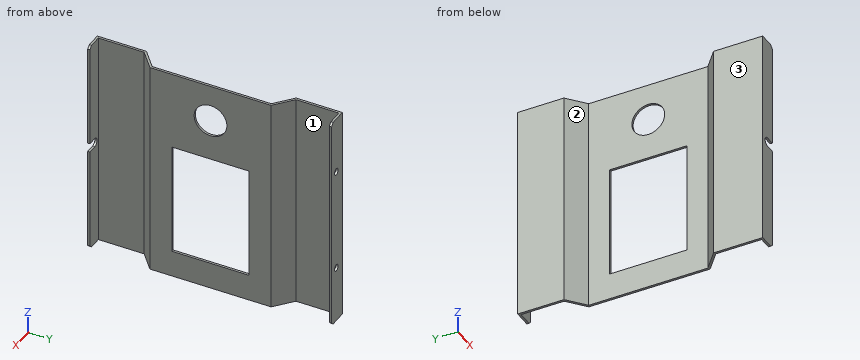
```python
from build123d import *

# Parameters (mm, degrees)
EXTRUDE_THIN1_DEPTH = 73.5
SKETCH2_W           = 76
SKETCH2_H           = 52
CUT_EXTRUDE1_DEPTH  = 10
CHAMFER1_SIZE       = 2
CUT_EXTRUDE3_DEPTH  = 5
SKETCH7_R           = 11
CUT_EXTRUDE4_DEPTH  = 10
SKETCH8_R           = 2.25
CUT_EXTRUDE5_DEPTH  = 10


with BuildPart() as part:
    # Sketch1 → Extrude-Thin1 (new, symmetric)
    with BuildSketch(Plane.XY):
        Polygon((12, 0), (0, 0), (0, 33), (12, 43.248968226), (12, 123.248968226), (0, 133.497936451), (0, 164.497936451), (13.5, 164.497936451), (13.5, 162.997936451), (1.5, 162.997936451), (1.5, 134.189445923), (13.5, 123.940477697), (13.5, 42.557458754), (1.5, 32.308490528), (1.5, 1.5), (12, 1.5), align=None)
    extrude(amount=EXTRUDE_THIN1_DEPTH, both=True)

    # Sketch2 → Cut-Extrude1 (cut)
    with BuildSketch(Plane.ZY.offset(-12)):
        with Locations((-17.5, 83.248968226)):
            Rectangle(SKETCH2_W, SKETCH2_H)
    extrude(amount=-CUT_EXTRUDE1_DEPTH, mode=Mode.SUBTRACT)

    # Chamfer1
    chamfer1_edges = [part.edges().sort_by_distance(p)[0] for p in [
        (13.5, 163.747936451, -73.5),
        (12, 0.75, -73.5),
        (13.5, 163.747936451, 73.5),
        (12, 0.75, 73.5),
    ]]
    chamfer(chamfer1_edges, length=CHAMFER1_SIZE)

    # Sketch6 → Cut-Extrude3 (cut)
    with BuildSketch(Plane.XZ):
        with BuildLine():
            Line((6, 3), (12, 3))
            ThreePointArc((12, 3), (15, 0), (12, -3))
            Line((12, -3), (6, -3))
            ThreePointArc((6, -3), (3, 0), (6, 3))
        make_face()
    extrude(amount=-CUT_EXTRUDE3_DEPTH, mode=Mode.SUBTRACT)

    # Sketch7 → Cut-Extrude4 (cut)
    with BuildSketch(Plane.ZY.offset(-12)):
        with Locations(Location((48.5, 83.248968226, 0), (0, 0, 270))):
            Circle(SKETCH7_R)
    extrude(amount=-CUT_EXTRUDE4_DEPTH, mode=Mode.SUBTRACT)

    # Sketch8 → Cut-Extrude5 (cut)
    with BuildSketch(Plane(origin=(0, 164.497936451, 0), x_dir=(1, 0, 0), z_dir=(0, 1, 0))):
        with Locations(Location((7.5, 35, 0), (0, 0, 180))):
            Circle(SKETCH8_R)
    cut_extrude5 = extrude(amount=-CUT_EXTRUDE5_DEPTH, mode=Mode.SUBTRACT)

    # Mirror1: Cut-Extrude5 across plane
    add(cut_extrude5.mirror(Plane.XY), mode=Mode.SUBTRACT)


solid = part.part
```
Build history of the part. All positions in model axes, mm. Face numbers are marked on the shaded views. A direction names the side the tool comes from. Give positions to 0.01 mm unless a question says otherwise; leave off trailing zeros. Loops run counter-clockwise (first coordinate to the right, second up) from the corner with the lowest first, then second, coordinate; pieces in that order, holes last.
1) 3-axis set-ups, long thin cutter, end or side, ignore diameter. For the marked faces 1, 2 and 3: which of +Z, -Z, +X, -X, +Y, -Y reach the whole face in a straight line?
Values follow:
face 1: +Z, -Z, +X
face 2: +Z, -Z, -X
face 3: +Z, -Z, -X, +Y, -Y
2) Band-saw the part on B-B on y = 61.5. List the corners of the cut face in (x, z), then the cut area to 4 significant figures.
Values follow:
outline: (12, -73.5) - (13.5, -73.5) - (13.5, -55.5) - (12, -55.5) - close; (12, 20.5) - (13.5, 20.5) - (13.5, 73.5) - (12, 73.5) - close
area: 106.5 mm2
3) Probe line 1 along Z through (x, y) = (7.5, 163.85); line 2 along Y through (x, z) = (4.5, 1); line 3 along Y through (x, z) = (2, -38). List the from-to ranges inside material, lowest first.
Values follow:
line 1: z = -73.5 to -37.25, -32.75 to 32.75, 37.25 to 73.5
line 2: y = 34.87 to 36.84, 129.65 to 131.63, 163 to 164.5
line 3: y = 0 to 1.5, 32.74 to 34.71, 131.79 to 133.76, 163 to 164.5
4) Band-saw the part on A-A on z = 0. List the corners of the cut face in (x, y).
Values follow:
outline: (0, 0) - (3, 0) - (3, 1.5) - (1.5, 1.5) - (1.5, 32.31) - (13.5, 42.56) - (13.5, 57.25) - (12, 57.25) - (12, 43.25) - (0, 33) - close; (0, 133.5) - (12, 123.25) - (12, 109.25) - (13.5, 109.25) - (13.5, 123.94) - (1.5, 134.19) - (1.5, 163) - (13.5, 163) - (13.5, 164.5) - (0, 164.5) - close
5) Band-saw the part on D-D on z = 24.5. List the corners of the cut face in (x, y).
Values follow:
outline: (0, 0) - (12, 0) - (12, 1.5) - (1.5, 1.5) - (1.5, 32.31) - (13.5, 42.56) - (13.5, 123.94) - (1.5, 134.19) - (1.5, 163) - (13.5, 163) - (13.5, 164.5) - (0, 164.5) - (0, 133.5) - (12, 123.25) - (12, 43.25) - (0, 33) - close
6) Drop flat-ended pins along their axis: P1, Ø1.6, axis at y = 1, z = -43, coming from the +X side; P2, Ø10, axis at y = 84.5, z = -46, coming from the -X side; P3, Ø24, axis at y = 68.5, z = -2.5, coming from the -X side; P4, Ø0.8, axis at x = 13, z = -14.5, coming from the -Y side. Give the stop position or say it passes through.
Values follow:
P1: stops at x = 12
P2: passes through
P3: stops at x = 12
P4: stops at y = 41.79
7) Band-saw the part on C-C on z = -22. List the corners of the cut face in (x, y), then the cut area to 3 significant figures.
Values follow:
outline: (0, 0) - (12, 0) - (12, 1.5) - (1.5, 1.5) - (1.5, 32.31) - (13.5, 42.56) - (13.5, 57.25) - (12, 57.25) - (12, 43.25) - (0, 33) - close; (0, 133.5) - (12, 123.25) - (12, 109.25) - (13.5, 109.25) - (13.5, 123.94) - (1.5, 134.19) - (1.5, 163) - (13.5, 163) - (13.5, 164.5) - (0, 164.5) - close
area: 219 mm2
